Can you work these out from the model? Positions are in its coordinate system, mm. A direction names the side the tool comes from. Give positions to 0.01 mm unless a question says otherwise; leave off trailing zeros. Write each loop counter-clockwise with the first axis right and the second up, starting at its lowest first coordinate (ties: lowest second). Pieces come first, ordered by that corner, then holes.
from build123d import *

# Parameters (mm, degrees)
SKETCH1_R           = 48.5
BOSS_EXTRUDE1_DEPTH = 16
SKETCH2_R           = 3.35
CUT_EXTRUDE1_DEPTH  = 81.796039507
M8_TAPPED_HOLE2_D   = 6.8
CUT_EXTRUDE2_START  = -2
SKETCH5_R           = 50
CUT_EXTRUDE2_DEPTH  = 2
CHAMFER1_SIZE       = 1


with BuildPart() as part:
    # Sketch1 → Boss-Extrude1 (new body)
    with BuildSketch(Plane.XY):
        with BuildLine():
            Line((-46, 56), (46, 56))
            ThreePointArc((46, 56), (53.071067812, 53.071067812), (56, 46))
            Line((56, 46), (56, -46))
            ThreePointArc((56, -46), (53.071067812, -53.071067812), (46, -56))
            Line((46, -56), (-46, -56))
            ThreePointArc((-46, -56), (-53.071067812, -53.071067812), (-56, -46))
            Line((-56, -46), (-56, 46))
            ThreePointArc((-56, 46), (-53.071067812, 53.071067812), (-46, 56))
        make_face()
        Circle(SKETCH1_R, mode=Mode.SUBTRACT)
    extrude(amount=BOSS_EXTRUDE1_DEPTH)

    # Sketch2 → Cut-Extrude1 (cut, through all)
    with BuildSketch(Plane.XY.offset(16)):
        with Locations((-42.5, 42.5)):
            Circle(SKETCH2_R)
        with Locations((42.5, 42.5)):
            Circle(SKETCH2_R)
        with Locations((42.5, -42.5)):
            Circle(SKETCH2_R)
        with Locations((-42.5, -42.5)):
            Circle(SKETCH2_R)
    extrude(amount=-CUT_EXTRUDE1_DEPTH, mode=Mode.SUBTRACT)

    # M8 Tapped Hole2 (through all)
    with Locations(Plane.XY.offset(16)):
        with Locations((-42.5, 42.5), (42.5, 42.5), (42.5, -42.5), (-42.5, -42.5)):
            Hole(M8_TAPPED_HOLE2_D / 2)

    # Sketch5 → Cut-Extrude2 (cut)
    with BuildSketch(Plane.XY.offset(16).offset(CUT_EXTRUDE2_START)):
        with BuildLine():
            Line((56, -46), (56, 46))
            ThreePointArc((56, 46), (53.071067812, 53.071067812), (46, 56))
            Line((46, 56), (-46, 56))
            ThreePointArc((-46, 56), (-53.071067812, 53.071067812), (-56, 46))
            Line((-56, 46), (-56, -46))
            ThreePointArc((-56, -46), (-53.071067812, -53.071067812), (-46, -56))
            Line((-46, -56), (46, -56))
            ThreePointArc((46, -56), (53.071067812, -53.071067812), (56, -46))
        make_face()
        Circle(SKETCH5_R, mode=Mode.SUBTRACT)
    extrude(amount=CUT_EXTRUDE2_DEPTH, mode=Mode.SUBTRACT)

    # Chamfer1
    chamfer1_edges = [part.edges().sort_by_distance(p)[0] for p in [
        (56, 0, 0),
        (53.071067812, -53.071067812, 0),
        (0, -56, 0),
        (-53.071067812, -53.071067812, 0),
        (-56, 0, 0),
        (-53.071067812, 53.071067812, 0),
        (0, 56, 0),
        (53.071067812, 53.071067812, 14),
        (56, 0, 14),
        (53.071067812, -53.071067812, 14),
        (0, -56, 14),
        (-53.071067812, -53.071067812, 14),
        (-56, 0, 14),
        (-53.071067812, 53.071067812, 14),
        (0, 56, 14),
        (53.071067812, 53.071067812, 0),
    ]]
    chamfer(chamfer1_edges, length=CHAMFER1_SIZE)


solid = part.part
(1) If I drill on L1, parallel to X at y = 1, z = 6.5; L2, parallel to Y at x = -42.5, z = 8; L3, parallel to Y at x = -42, z = 3, over which ranges is the centre line in solid material (lowest first)?
Returned:
L1: x = -56 to -48.49, 48.49 to 56
L2: y = -56 to -45.9, -39.1 to -23.37, 23.37 to 39.1, 45.9 to 56
L3: y = -56 to -45.86, -39.14 to -24.25, 24.25 to 39.14, 45.86 to 56
(2) For faces 1 (the face through (52.99, 53.15, 6.92)), 2 (the face through (-41, 29, 14)), which set-ups out of +Z, -Z, +X, -X, +Y, -Y let a thin tool reach every point of the face, with its end or its side?
Returned:
face 1: +Z, -Z, +X, +Y
face 2: +Z
(3) Imagine slicing it at B-B, the plane y = 11.5. Write out the boundary of the cut face in (x, z), plus the area to 3 significant figures.
Returned:
outline: (-56, 1) - (-55, 0) - (-47.12, 0) - (-47.12, 16) - (-48.66, 16) - (-48.66, 14) - (-55, 14) - (-56, 13) - close; (47.12, 0) - (55, 0) - (56, 1) - (56, 13) - (55, 14) - (48.66, 14) - (48.66, 16) - (47.12, 16) - close
area: 253 mm2
(4) If we mould it in two halves opening along X, with no side actions, what happens to faces 3 (the face through (-45.64, -43.8, 6.9)), 4 (the face through (-52.99, -53.15, 6.92)), 5 (the face through (-1, 56, 7))? For each: +X half, -X half, draft (parallel to the pull), parting line (faces both ways), or undercut.
Returned:
face 3: undercut
face 4: -X half
face 5: draft
(5) Imagine slicing it at C-C, the plane z = 3.75. Write out the boundary of the cut face in (x, y).
Returned:
outline: (-56, -46) arc R10 ccw to (-46, -56) - (46, -56) arc R10 ccw to (56, -46) - (56, 46) arc R10 ccw to (46, 56) - (-46, 56) arc R10 ccw to (-56, 46) - close; hole circle Ø97 at (0, 0); hole circle Ø6.8 at (-42.5, -42.5); hole circle Ø6.8 at (-42.5, 42.5); hole circle Ø6.8 at (42.5, -42.5); hole circle Ø6.8 at (42.5, 42.5)
(6) Will this pin go through, and if not, where does the flat tip stop? P1, Ø4, axis at x = -42.5, y = 42.5, coming from the +Z side.
Returned:
P1: passes through
(7) Imagine slicing it at D-D, the plane y = 40.5. Write out the boundary of the cut face in (x, z), plus the area to 3 significant figures.
Returned:
outline: (-56, 1) - (-55, 0) - (-45.25, 0) - (-45.25, 14) - (-55, 14) - (-56, 13) - close; (-39.75, 0) - (-26.68, 0) - (-26.68, 16) - (-29.32, 16) - (-29.32, 14) - (-39.75, 14) - close; (26.68, 0) - (39.75, 0) - (39.75, 14) - (29.32, 14) - (29.32, 16) - (26.68, 16) - close; (45.25, 0) - (55, 0) - (56, 1) - (56, 13) - (55, 14) - (45.25, 14) - close
area: 675 mm2
(8) Imagine slicing it at A-A, the plane x = -24.5. Write out the boundary of the cut face in (y, z).
Returned:
outline: (-56, 1) - (-55, 0) - (-41.86, 0) - (-41.86, 16) - (-43.59, 16) - (-43.59, 14) - (-55, 14) - (-56, 13) - close; (41.86, 0) - (55, 0) - (56, 1) - (56, 13) - (55, 14) - (43.59, 14) - (43.59, 16) - (41.86, 16) - close
